Input: part model. Units: mm. Frame: model coordinates. Face numbers are marked on the shaded views. A direction names the side the tool comes from. Round coordinates to 2 decimals unless told otherwise and drop trailing zeros. Loops run counter-clockwise (first coordinate to the right, second up) from the corner with the lowest first, then second, coordinate; pieces in that order, holes last. Notation, with made-up numbers: (52.5, 30.25) -> (56.5, 30.25) arc R14 ccw to (56.5, 42.25) -> close; hole circle Ø3 at (40, 21.5). An arc over 180 degrees is marked (long way). Answer as a JSON object with one key per item and string values.
```python
from build123d import *

# Parameters (mm, degrees)
SKETCH1_W                                           = 13
SKETCH1_H                                           = 25
BOSS_EXTRUDE1_DEPTH                                 = 10
CUT_EXTRUDE1_DEPTH                                  = 18.277152543
CUT_EXTRUDE1_DEPTH_BACK                             = 18.277152543
SKETCH2_W                                           = 2.5
SKETCH2_H                                           = 10
FILLET1_R                                           = 0.5
FILLET2_R                                           = 1
SKETCH8_W                                           = 6
SKETCH8_H                                           = 32.589216013
CUT_EXTRUDE4_DEPTH                                  = 1
SKETCH21_W                                          = 10
SKETCH21_H                                          = 30.602707306
CUT_EXTRUDE11_DEPTH                                 = 1
SKETCH25_W                                          = 13.801043237
SKETCH25_H                                          = 15.676526687
CUT_EXTRUDE13_DEPTH                                 = 2
FILLET3_R                                           = 1
CBORE_FOR_M3_HEX_SOCKET_HEAD_CAP_SCREW2_D           = 3.4
CBORE_FOR_M3_HEX_SOCKET_HEAD_CAP_SCREW2_CBORE_D     = 6.5
CBORE_FOR_M3_HEX_SOCKET_HEAD_CAP_SCREW2_CBORE_DEPTH = 5.4
BOSS_EXTRUDE4_START                                 = 6
BOSS_EXTRUDE4_DEPTH                                 = 6
CUT_EXTRUDE15_REACH                                 = 26.109
SKETCH33_W                                          = 10.378798484
SKETCH33_H                                          = 20
SKETCH34_W                                          = 9.92103125
SKETCH34_H                                          = 19.736261401
CUT_EXTRUDE16_DEPTH                                 = 2.5
BOSS_EXTRUDE5_START                                 = 2
BOSS_EXTRUDE5_DEPTH                                 = 2
M3_TAPPED_HOLE1_D                                   = 2.5
M3_TAPPED_HOLE1_DEPTH                               = 7.5
M3_TAPPED_HOLE1_TIP                                 = 0.751075774
M3_TAPPED_HOLE2_D                                   = 2.5
M3_TAPPED_HOLE2_DEPTH                               = 7.5
M3_TAPPED_HOLE2_TIP                                 = 0.751075774
SKETCH41_R                                          = 1
CUT_EXTRUDE17_DEPTH                                 = 5


with BuildPart() as part:
    # Sketch1 → Boss-Extrude1 (new body)
    with BuildSketch(Plane.XY):
        Rectangle(SKETCH1_W, SKETCH1_H)
    extrude(amount=BOSS_EXTRUDE1_DEPTH)

    # Sketch2 → Cut-Extrude1 (cut, two sides: drawn at the far end of the back side and taken through both)
    with BuildSketch(Plane.XY.offset(10).offset(-CUT_EXTRUDE1_DEPTH_BACK)):
        with Locations((-5.25, 7.5)):
            Rectangle(SKETCH2_W, SKETCH2_H)
        with Locations((5.25, 7.5)):
            Rectangle(SKETCH2_W, SKETCH2_H)
    extrude(amount=CUT_EXTRUDE1_DEPTH + CUT_EXTRUDE1_DEPTH_BACK, mode=Mode.SUBTRACT)

    # Fillet1
    fillet1_edges = [part.edges().sort_by_distance(p)[0] for p in [
        (-6.5, 2.5, 5),
        (-4, 2.5, 5),
        (6.5, 2.5, 5),
        (4, 2.5, 5),
        (6.5, -12.5, 5),
        (-6.5, -12.5, 5),
    ]]
    fillet(fillet1_edges, radius=FILLET1_R)

    # Fillet2
    fillet2_edges = [part.edges().sort_by_distance(p)[0] for p in [
        (-4, 12.5, 5),
        (4, 12.5, 5),
    ]]
    fillet(fillet2_edges, radius=FILLET2_R)

    # Sketch8 → Cut-Extrude4 (cut)
    with BuildSketch(Plane(origin=(0, 0, 0), x_dir=(-1, 0, 0), z_dir=(0, 0, -1))):
        with Locations((0, -3.794608007)):
            Rectangle(SKETCH8_W, SKETCH8_H)
    extrude(amount=-CUT_EXTRUDE4_DEPTH, mode=Mode.SUBTRACT)

    # Sketch21 → Cut-Extrude11 (cut)
    with BuildSketch(Plane.XY.offset(10)):
        with Locations((0, 4.301353653)):
            Rectangle(SKETCH21_W, SKETCH21_H)
    extrude(amount=-CUT_EXTRUDE11_DEPTH, mode=Mode.SUBTRACT)

    # Sketch25 → Cut-Extrude13 (cut)
    with BuildSketch(Plane.XY.offset(9)):
        with Locations((-1.252110778, 12.838263344)):
            Rectangle(SKETCH25_W, SKETCH25_H)
    extrude(amount=-CUT_EXTRUDE13_DEPTH, mode=Mode.SUBTRACT)

    # Fillet3
    fillet3_edges = [part.edges().sort_by_distance(p)[0] for p in [
        (4, 5, 8),
        (-4, 5, 8),
    ]]
    fillet(fillet3_edges, radius=FILLET3_R)

    # CBORE for M3 Hex Socket Head Cap Screw2 (through all)
    with Locations(Plane.XY.offset(9)):
        with Locations((0, 9)):
            CounterBoreHole(CBORE_FOR_M3_HEX_SOCKET_HEAD_CAP_SCREW2_D / 2, CBORE_FOR_M3_HEX_SOCKET_HEAD_CAP_SCREW2_CBORE_D / 2, CBORE_FOR_M3_HEX_SOCKET_HEAD_CAP_SCREW2_CBORE_DEPTH)

    # Sketch31 → Boss-Extrude4 (add)
    with BuildSketch(Plane.XY.offset(10).offset(BOSS_EXTRUDE4_START)):
        with BuildLine():
            Line((-5, -11), (-5, 2.5))
            Line((-5, 2.5), (-6, 2.5))
            ThreePointArc((-6, 2.5), (-6.353553391, 2.353553391), (-6.5, 2))
            Line((-6.5, 2), (-6.5, -12))
            ThreePointArc((-6.5, -12), (-6.353553391, -12.353553391), (-6, -12.5))
            Line((-6, -12.5), (6, -12.5))
            ThreePointArc((6, -12.5), (6.353553391, -12.353553391), (6.5, -12))
            Line((6.5, -12), (6.5, 2))
            ThreePointArc((6.5, 2), (6.353553391, 2.353553391), (6, 2.5))
            Line((6, 2.5), (5, 2.5))
            Line((5, 2.5), (5, -11))
            Line((5, -11), (-5, -11))
        make_face()
    extrude(amount=-BOSS_EXTRUDE4_DEPTH)

    # Cut-Extrude15: up to this face of the body (flat: up to its plane)
    cut_extrude15_end = Plane(part.part.faces().sort_by_distance((-4, 7.12804878, 3.646341463))[0])
    # Sketch33 → Cut-Extrude15 (cut, up to the picked face)
    with BuildSketch(Plane.ZY.offset(6.5), mode=Mode.PRIVATE) as cut_extrude15_sk1:
        with Locations((3.310600758, -6.5)):
            Rectangle(SKETCH33_W, SKETCH33_H)
    cut_extrude15_tool1 = split(extrude(cut_extrude15_sk1.sketch, amount=-CUT_EXTRUDE15_REACH, mode=Mode.PRIVATE), bisect_by=cut_extrude15_end, keep=Keep.BOTH, mode=Mode.PRIVATE)
    add(cut_extrude15_tool1.solids().sort_by(Axis((-6.5, -6.5, 3.310601), (1, 0, 0)))[0], mode=Mode.SUBTRACT)

    # Sketch34 → Cut-Extrude16 (cut)
    with BuildSketch(Plane(origin=(6.5, 0, 0), x_dir=(0, 0, -1), z_dir=(1, 0, 0))):
        with Locations((-3.539484375, -6.368130701)):
            Rectangle(SKETCH34_W, SKETCH34_H)
    extrude(amount=-CUT_EXTRUDE16_DEPTH, mode=Mode.SUBTRACT)

    # Sketch36 → Boss-Extrude5 (add)
    with BuildSketch(Plane.XY.offset(9).offset(BOSS_EXTRUDE5_START)):
        with BuildLine():
            Line((-5, 2.5), (-5, -11))
            Line((-5, -11), (5, -11))
            Line((5, -11), (5, 2.5))
            Line((5, 2.5), (4.5, 2.5))
            ThreePointArc((4.5, 2.5), (4.146446609, 2.646446609), (4, 3))
            Line((4, 3), (4, 4))
            ThreePointArc((4, 4), (3.707106781, 4.707106781), (3, 5))
            Line((3, 5), (-3, 5))
            ThreePointArc((-3, 5), (-3.707106781, 4.707106781), (-4, 4))
            Line((-4, 4), (-4, 3))
            ThreePointArc((-4, 3), (-4.146446609, 2.646446609), (-4.5, 2.5))
            Line((-4.5, 2.5), (-5, 2.5))
        make_face()
    extrude(amount=-BOSS_EXTRUDE5_DEPTH)

    # M3 Tapped Hole1
    with Locations(Plane.XY.offset(11)):
        with Locations((0, -5.5)):
            Hole(M3_TAPPED_HOLE1_D / 2, depth=M3_TAPPED_HOLE1_DEPTH)
            with Locations((0, 0, -(M3_TAPPED_HOLE1_DEPTH + M3_TAPPED_HOLE1_TIP / 2))):  # 118° drill point
                Cone(0, M3_TAPPED_HOLE1_D / 2, M3_TAPPED_HOLE1_TIP, mode=Mode.SUBTRACT)

    # M3 Tapped Hole2
    with Locations(Plane(origin=(0, -12.5, 0), x_dir=(-1, 0, 0), z_dir=(0, -1, 0))):
        with Locations((0, -13.5)):
            Hole(M3_TAPPED_HOLE2_D / 2, depth=M3_TAPPED_HOLE2_DEPTH)
            with Locations((0, 0, -(M3_TAPPED_HOLE2_DEPTH + M3_TAPPED_HOLE2_TIP / 2))):  # 118° drill point
                Cone(0, M3_TAPPED_HOLE2_D / 2, M3_TAPPED_HOLE2_TIP, mode=Mode.SUBTRACT)

    # Sketch41 → Cut-Extrude17 (cut)
    with BuildSketch(Plane.XY.offset(16)):
        with Locations((-5, -11)):
            Circle(SKETCH41_R)
        with Locations((5, -11)):
            Circle(SKETCH41_R)
    extrude(amount=-CUT_EXTRUDE17_DEPTH, mode=Mode.SUBTRACT)


solid = part.part
```
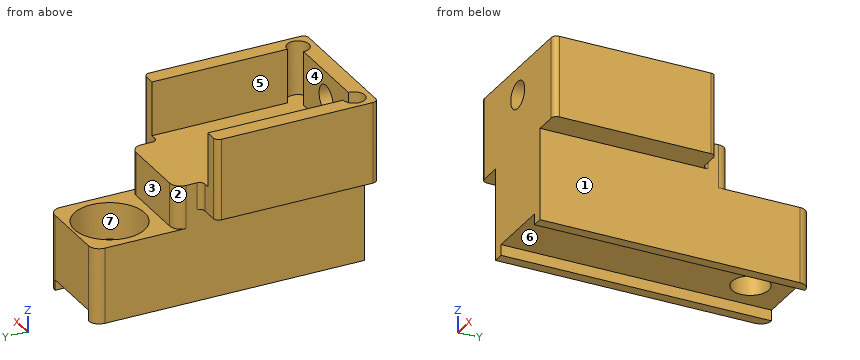
1) Section B-B, the plane z = 13. Output: boundary loops of the cut face in (x, y), plus the area to 3 significant figures.
Output:
{"outline": "(-6.5, -12) arc R0.5 ccw to (-6, -12.5) -> (-1.15, -12.5) -> (-1.15, -11) -> (-4, -11) arc R1 cw (long way) to (-5, -10) -> (-5, 2.5) -> (-6, 2.5) arc R0.5 ccw to (-6.5, 2) -> close; (1.15, -12.5) -> (6, -12.5) arc R0.5 ccw to (6.5, -12) -> (6.5, 2) arc R0.5 ccw to (6, 2.5) -> (5, 2.5) -> (5, -10) arc R1 cw (long way) to (4, -11) -> (1.15, -11) -> close", "area": "51.6 mm^2"}
2) Section A-A, the plane z = 5. Output: boundary loops of the cut face in (x, y), plus the area to 3 significant figures.
Output:
{"outline": "(-4, -12.5) -> (4, -12.5) -> (4, 11.5) arc R1 ccw to (3, 12.5) -> (-3, 12.5) arc R1 ccw to (-4, 11.5) -> close; hole circle Ø6.5 at (0, 9); hole circle Ø2.5 at (0, -5.5)", "area": "161 mm^2"}
3) Reachability of the marked faces 5, 6 and 7 from +Z, -Z, +X, -X, +Y, -Y: full face, straight path, thin tool, end or side. Return the list, or none.
Output:
{"face 5": "+Z, +Y", "face 6": "-Z, +Y, -Y", "face 7": "+Z"}
4) Section C-C, the plane x = -0.5. Count the separate pieces of the cut face and the enclosed holes in it, plus the area to 3 significant figures.
Output:
{"separate pieces": "3", "enclosed holes": "0", "area": "176 mm^2"}
5) Draft query along X for the marked faces 1, 2, 3 and 4. Return one class per face: +X half, -X half, draft (parallel to the pull), parting line (faces both ways), or undercut.
Output:
{"face 1": "+X half", "face 2": "-X half", "face 3": "draft", "face 4": "undercut"}
6) Contact query for flat-ended pins moving along their axis: P1, Ø7, axis at x = -1.5, y = 10, coming from the +Z side; P2, Ø4, axis at x = 1, z = 12.5, coming from the +Y side; P3, Ø4, axis at x = -4.5, y = 6, coming from the +Z side; P4, Ø9, axis at y = -4, z = 8, coming from the +X side. Output: stop coordinate, or through.
Output:
{"P1": "stops at z = 7", "P2": "stops at y = 5", "P3": "stops at z = 11", "P4": "stops at x = 6.5"}
7) Ray query, probe 1 along Y at (x, z) = (0, 5.75); probe 2 along X at (y, z) = (-6.25, 12.25); probe 3 along Y at (x, z) = (0, 8.5). Return the intervals inside material, ascending.
Output:
{"probe 1": "y = -12.5 to -6.75, -4.25 to 5.75, 12.25 to 12.5", "probe 2": "x = -6.5 to -5, 5 to 6.5", "probe 3": "y = -12.5 to -6.75, -4.25 to 5"}
